For this review, use the dimensioned drawing (mm, ordinates from the lowest corner) and the shaded views. Give positions to 0.01 mm unless a question says otherwise; leave off trailing zeros. Order: outer loops, then holes, each group sorted by start corner. A loop starts at its lowest first (then second) coordinate and runs counter-clockwise, first axis right, second up. Notation, with made-up numbers: (47, 81.25) -> (80, 81.25) arc R26 ccw to (80, 104.25) -> close; hole circle Ø6 at (-34.75, -0.5). An arc over 180 degrees is marked (long way). Return JSON: item names as keys, results as strings.
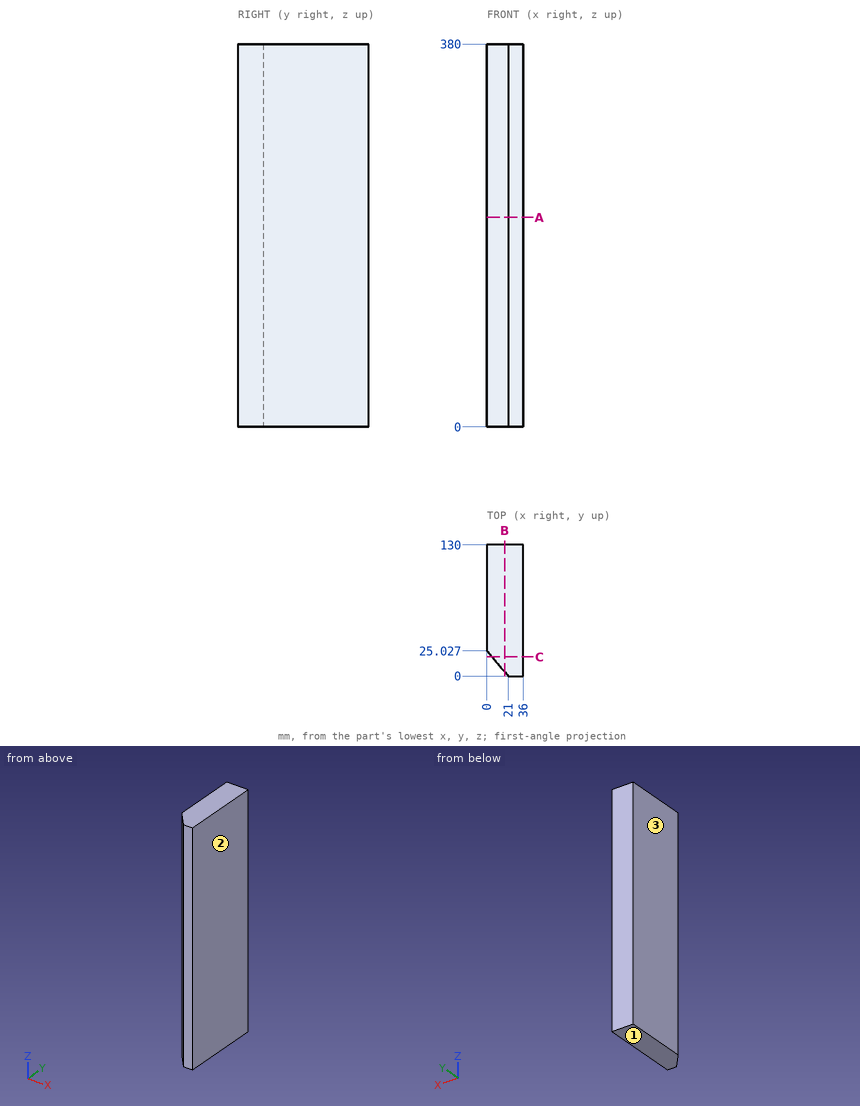
Item 1: Add section B-B (x = 17.5). Give the boundary of the cut face in (y, z), plus the area to 3 significant figures.
Result set:
{"outline": "(4.17, 0) -> (130, 0) -> (130, 380) -> (4.17, 380) -> close", "area": "47,800 mm^2"}
Item 2: Wall thickness on L1, parallel to Y at x = 5, z = 255; L2, parallel to X at y = 19.5, z = 67; L3, parallel to Y at x = 8.5, z = 316: over which ranges is each line inside the solid? List them lowest first. Write a range as [from, to].
Result set:
{"L1": "y = [19.07, 130]", "L2": "x = [4.64, 36]", "L3": "y = [14.9, 130]"}
Item 3: Add section A-A (z = 208). Give the boundary of the cut face in (x, y), plus the area to 3 significant figures.
Result set:
{"outline": "(0, 25.03) -> (21, 0) -> (36, 0) -> (36, 130) -> (0, 130) -> close", "area": "4,420 mm^2"}
Item 4: Mouldability with a two-part tool opening along X and no side actions: class the marked faces 1, 2 and 3 as released by +X, released by -X, zero draft, split by the parting line, or undercut.
Result set:
{"face 1": "zero draft", "face 2": "released by +X", "face 3": "released by -X"}
Item 5: Add section C-C (y = 19). Give the boundary of the cut face in (x, z), plus the area to 3 significant figures.
Result set:
{"outline": "(5.06, 0) -> (36, 0) -> (36, 380) -> (5.06, 380) -> close", "area": "11,800 mm^2"}
Item 6: For pin 1 (1.5 mm diameter, centred on x = 13, z = 285, fed in from -Y); pin 2 (6 mm diameter, centred on x = 6.5, y = 104, fed in from -Z); pin 3 (1 mm diameter, centred on x = 4, z = 236.5, fed in from -Y), all flat-tipped, find the tip position at first contact; note any pin that passes through.
Result set:
{"pin 1": "stops at y = 8.64", "pin 2": "stops at z = 0", "pin 3": "stops at y = 19.66"}
